Can you work these out from the model? Positions are in its coordinate system, mm. A direction names the side the tool comes from. Coordinates: 2 decimals unless noted, no trailing zeros. Loops run counter-clockwise (first coordinate to the right, second up) from the corner with the lowest first, then second, coordinate; pieces in that order, holes last. Notation, with made-up numbers: M 37,53 L 45,53 A13 ccw 45,73 Z; hole C 42,69 d5. An arc over 180 degrees is marked long. Return JSON: item names as keys, results as strings. Group by question number.
```python
from build123d import *

# Parameters (mm, degrees)
SKETCH4_R           = 1.25
BOSS_EXTRUDE3_DEPTH = 100
SCALE_1_SCALE       = 0.7
SKETCH5_R           = 0.875
BOSS_EXTRUDE4_DEPTH = 20


with BuildPart() as part:
    # Sketch4 → Boss-Extrude3 (new body)
    with BuildSketch(Plane.XY):
        with BuildLine():
            Line((-1.5, 7.5), (-7.2, 7.5))
            ThreePointArc((-7.2, 7.5), (-7.412132034, 7.412132034), (-7.5, 7.2))
            Line((-7.5, 7.2), (-7.5, 1.5))
            Line((-7.5, 1.5), (-6.5, 1.5))
            Line((-6.5, 1.5), (-6.5, 2.9))
            Line((-6.5, 2.9), (-4, 2.9))
            Line((-4, 2.9), (-4, 1.5))
            Line((-4, 1.5), (-2.5, 1.5))
            Line((-2.5, 1.5), (-2.5, -1.5))
            Line((-2.5, -1.5), (-4, -1.5))
            Line((-4, -1.5), (-4, -2.9))
            Line((-4, -2.9), (-6.5, -2.9))
            Line((-6.5, -2.9), (-6.5, -1.5))
            Line((-6.5, -1.5), (-7.5, -1.5))
            Line((-7.5, -1.5), (-7.5, -7.2))
            ThreePointArc((-7.5, -7.2), (-7.412132034, -7.412132034), (-7.2, -7.5))
            Line((-7.2, -7.5), (-1.5, -7.5))
            Line((-1.5, -7.5), (-1.5, -6.5))
            Line((-1.5, -6.5), (-2.9, -6.5))
            Line((-2.9, -6.5), (-2.9, -4))
            Line((-2.9, -4), (-1.5, -4))
            Line((-1.5, -4), (-1.5, -2.5))
            Line((-1.5, -2.5), (1.5, -2.5))
            Line((1.5, -2.5), (1.5, -4))
            Line((1.5, -4), (2.9, -4))
            Line((2.9, -4), (2.9, -6.5))
            Line((2.9, -6.5), (1.5, -6.5))
            Line((1.5, -6.5), (1.5, -7.5))
            Line((1.5, -7.5), (7.2, -7.5))
            ThreePointArc((7.2, -7.5), (7.412132034, -7.412132034), (7.5, -7.2))
            Line((7.5, -7.2), (7.5, -1.5))
            Line((7.5, -1.5), (6.5, -1.5))
            Line((6.5, -1.5), (6.5, -2.9))
            Line((6.5, -2.9), (4, -2.9))
            Line((4, -2.9), (4, -1.5))
            Line((4, -1.5), (2.5, -1.5))
            Line((2.5, -1.5), (2.5, 1.5))
            Line((2.5, 1.5), (4, 1.5))
            Line((4, 1.5), (4, 2.9))
            Line((4, 2.9), (6.5, 2.9))
            Line((6.5, 2.9), (6.5, 1.5))
            Line((6.5, 1.5), (7.5, 1.5))
            Line((7.5, 1.5), (7.5, 7.2))
            ThreePointArc((7.5, 7.2), (7.412132034, 7.412132034), (7.2, 7.5))
            Line((7.2, 7.5), (1.5, 7.5))
            Line((1.5, 7.5), (1.5, 6.5))
            Line((1.5, 6.5), (2.9, 6.5))
            Line((2.9, 6.5), (2.9, 4))
            Line((2.9, 4), (1.5, 4))
            Line((1.5, 4), (1.5, 2.5))
            Line((1.5, 2.5), (-1.5, 2.5))
            Line((-1.5, 2.5), (-1.5, 4))
            Line((-1.5, 4), (-2.9, 4))
            Line((-2.9, 4), (-2.9, 6.5))
            Line((-2.9, 6.5), (-1.5, 6.5))
            Line((-1.5, 6.5), (-1.5, 7.5))
        make_face()
        with Locations((-5, -5)):
            Circle(SKETCH4_R, mode=Mode.SUBTRACT)
        Circle(SKETCH4_R, mode=Mode.SUBTRACT)
        with Locations((5, -5)):
            Circle(SKETCH4_R, mode=Mode.SUBTRACT)
        with Locations((-5, 5)):
            Circle(SKETCH4_R, mode=Mode.SUBTRACT)
        with Locations((5, 5)):
            Circle(SKETCH4_R, mode=Mode.SUBTRACT)
    extrude(amount=BOSS_EXTRUDE3_DEPTH)


with BuildPart() as part_1:
    # Scale 1: scaled about (0, 0, 0)
    add(part.part.scale(SCALE_1_SCALE))

    # Sketch5 → Boss-Extrude4 (add)
    with BuildSketch(Plane.XY.offset(70)):
        with BuildLine():
            Line((-1.05, 5.25), (-5.04, 5.25))
            ThreePointArc((-5.04, 5.25), (-5.188492424, 5.188492424), (-5.25, 5.04))
            Line((-5.25, 5.04), (-5.25, 1.05))
            Line((-5.25, 1.05), (-4.55, 1.05))
            Line((-4.55, 1.05), (-4.55, 2.03))
            Line((-4.55, 2.03), (-2.8, 2.03))
            Line((-2.8, 2.03), (-2.8, 1.05))
            Line((-2.8, 1.05), (-1.75, 1.05))
            Line((-1.75, 1.05), (-1.75, -1.05))
            Line((-1.75, -1.05), (-2.8, -1.05))
            Line((-2.8, -1.05), (-2.8, -2.03))
            Line((-2.8, -2.03), (-4.55, -2.03))
            Line((-4.55, -2.03), (-4.55, -1.05))
            Line((-4.55, -1.05), (-5.25, -1.05))
            Line((-5.25, -1.05), (-5.25, -5.04))
            ThreePointArc((-5.25, -5.04), (-5.188492424, -5.188492424), (-5.04, -5.25))
            Line((-5.04, -5.25), (-1.05, -5.25))
            Line((-1.05, -5.25), (-1.05, -4.55))
            Line((-1.05, -4.55), (-2.03, -4.55))
            Line((-2.03, -4.55), (-2.03, -2.8))
            Line((-2.03, -2.8), (-1.05, -2.8))
            Line((-1.05, -2.8), (-1.05, -1.75))
            Line((-1.05, -1.75), (1.05, -1.75))
            Line((1.05, -1.75), (1.05, -2.8))
            Line((1.05, -2.8), (2.03, -2.8))
            Line((2.03, -2.8), (2.03, -4.55))
            Line((2.03, -4.55), (1.05, -4.55))
            Line((1.05, -4.55), (1.05, -5.25))
            Line((1.05, -5.25), (5.04, -5.25))
            ThreePointArc((5.04, -5.25), (5.188492424, -5.188492424), (5.25, -5.04))
            Line((5.25, -5.04), (5.25, -1.05))
            Line((5.25, -1.05), (4.55, -1.05))
            Line((4.55, -1.05), (4.55, -2.03))
            Line((4.55, -2.03), (2.8, -2.03))
            Line((2.8, -2.03), (2.8, -1.05))
            Line((2.8, -1.05), (1.75, -1.05))
            Line((1.75, -1.05), (1.75, 1.05))
            Line((1.75, 1.05), (2.8, 1.05))
            Line((2.8, 1.05), (2.8, 2.03))
            Line((2.8, 2.03), (4.55, 2.03))
            Line((4.55, 2.03), (4.55, 1.05))
            Line((4.55, 1.05), (5.25, 1.05))
            Line((5.25, 1.05), (5.25, 5.04))
            ThreePointArc((5.25, 5.04), (5.188492424, 5.188492424), (5.04, 5.25))
            Line((5.04, 5.25), (1.05, 5.25))
            Line((1.05, 5.25), (1.05, 4.55))
            Line((1.05, 4.55), (2.03, 4.55))
            Line((2.03, 4.55), (2.03, 2.8))
            Line((2.03, 2.8), (1.05, 2.8))
            Line((1.05, 2.8), (1.05, 1.75))
            Line((1.05, 1.75), (-1.05, 1.75))
            Line((-1.05, 1.75), (-1.05, 2.8))
            Line((-1.05, 2.8), (-2.03, 2.8))
            Line((-2.03, 2.8), (-2.03, 4.55))
            Line((-2.03, 4.55), (-1.05, 4.55))
            Line((-1.05, 4.55), (-1.05, 5.25))
        make_face()
        with Locations((3.5, -3.5)):
            Circle(SKETCH5_R, mode=Mode.SUBTRACT)
        with Locations((-3.5, -3.5)):
            Circle(SKETCH5_R, mode=Mode.SUBTRACT)
        with Locations((-3.5, 3.5)):
            Circle(SKETCH5_R, mode=Mode.SUBTRACT)
        with Locations((3.5, 3.5)):
            Circle(SKETCH5_R, mode=Mode.SUBTRACT)
        Circle(SKETCH5_R, mode=Mode.SUBTRACT)
    extrude(amount=BOSS_EXTRUDE4_DEPTH)


solid = part_1.part
```
1) If we mould it in two halves opening along X, with no side actions, what happens to faces 1 (the face through (0.808, -0.335, 44.37)), 2 (the face through (-1.75, 0, 44)), 3 (the face through (3, 5.25, 44))? For each: +X half, -X half, draft (parallel to the pull), parting line (faces both ways), or undercut.
2) If I drill on line 1 (Y direction, x = -3.5, z = 25) (3 decimals); line 2 (Y direction, x = 1.25, z = 6); line 3 (Y direction, x = -4.5, z = 45), over which ranges is the centre line in solid material (lowest first)? Write a range as from..to.
3) Suppose I cut it at B-B, the plane z = 82. Give the number of separate pieces and of enclosed holes in the cut face, then the cut area to 3 significant figures.
4) Suppose I cut it at A-A, the plane y = 0. List the corners of the cut face in (x, z) for me (3 decimals).
5) For faces 4 (the face through (2.03, -4, 44)), 5 (the face through (1.75, 0, 44)), 6 (the face through (0, -1.75, 44)), which set-ups out of +Z, -Z, +X, -X, +Y, -Y let a thin tool reach every point of the face, with its end or its side?
Returned:
{
 "1": {"face 1": "undercut", "face 2": "-X half", "face 3": "draft"},
 "2": {"line 1": "y = -5.25..-4.375, -2.625..-2.03, 2.03..2.625, 4.375..5.25", "line 2": "y = -5.25..-4.55, -2.8..2.8, 4.55..5.25", "line 3": "y = -5.25..-2.03, 2.03..5.25"},
 "3": {"separate pieces": "1", "enclosed holes": "5", "area": "55.1 mm²"},
 "4": {"outline": "M -1.75,0 L -0.875,0 L -0.875,90 L -1.75,90 Z; M 0.875,0 L 1.75,0 L 1.75,90 L 0.875,90 Z"},
 "5": {"face 4": "+Z, -Z", "face 5": "+Z, -Z, +X", "face 6": "+Z, -Z, -Y"}
}
